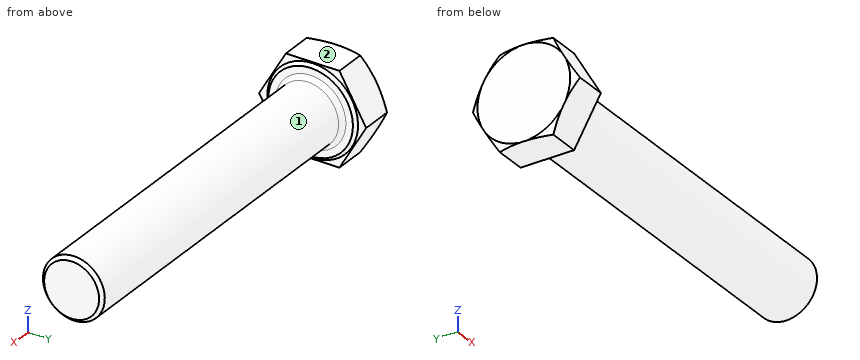
```python
from build123d import *

# Parameters (mm, degrees)
BOSS_EXTRUDE1_DEPTH = 7.5
SKETCH4_R           = 20.03
SKETCH4_R_2         = 9
CUT_EXTRUDE1_DEPTH  = 0.9375
CUT_EXTRUDE1_DRAFT  = -60
CHAMFER2_SIZE       = 0.666666667


with BuildPart() as part:
    # Sketch3 → Boss-Extrude1 (new body)
    with BuildSketch(Plane(origin=(0, 0, 0), x_dir=(0, 0, -1), z_dir=(1, 0, 0))):
        Polygon((9, 5.196152423), (0, 10.392304845), (-9, 5.196152423), (-9, -5.196152423), (0, -10.392304845), (9, -5.196152423), align=None)
    extrude(amount=BOSS_EXTRUDE1_DEPTH)


with BuildPart() as cut_extrude1_tool:
    # Sketch4 → Cut-Extrude1 (with draft: the straight prism first)
    with BuildSketch(Plane.ZY):
        Circle(SKETCH4_R)
        Circle(SKETCH4_R_2, mode=Mode.SUBTRACT)
    extrude(amount=-CUT_EXTRUDE1_DEPTH)
    # Cut-Extrude1: the draft: its side faces are tilted about the plane it starts from
    cut_extrude1_sides = [cut_extrude1_tool.faces().sort_by_distance(p)[0] for p in [
        (0.46875, 0, -20.03),
        (0.46875, 0, -9),
    ]]
    draft(cut_extrude1_sides, Plane.ZY, CUT_EXTRUDE1_DRAFT)


with BuildPart() as part_1:
    add(part.part)

    # Cut-Extrude1: cut by cut_extrude1_tool
    add(cut_extrude1_tool.part, mode=Mode.SUBTRACT)

    # Sketch5 → Revolve1 (revolve)
    with BuildSketch(Plane.XY, mode=Mode.PRIVATE) as revolve1_sk:
        with BuildLine():
            Line((8.35, 6), (77.5, 6))
            Line((77.5, 6), (77.5, 0))
            Line((77.5, 0), (7.5, 0))
            Line((7.5, 0), (7.5, 6.85))
            ThreePointArc((7.5, 6.85), (7.748959236, 6.248959236), (8.35, 6))
        make_face()
    revolve(revolve1_sk.sketch.rotate(Axis((7.5, 0, 0), (1, 0, 0)), 90), axis=Axis((7.5, 0, 0), (1, 0, 0)))

    # Chamfer2
    chamfer2_edges = [part_1.edges().sort_by_distance(p)[0] for p in [
        (77.5, 0, -6),
    ]]
    chamfer(chamfer2_edges, length=CHAMFER2_SIZE)

    # Sketch7 → Cut-Revolve1 (revolve, cut)
    with BuildSketch(Plane.XY, mode=Mode.PRIVATE) as cut_revolve1_sk:
        Polygon((7.5, 8.215), (6.9, 8.815), (6.9, 20.03), (7.5, 20.03), align=None)
    revolve(cut_revolve1_sk.sketch.rotate(Axis((0, 0, 0), (1, 0, 0)), 90), axis=Axis((0, 0, 0), (1, 0, 0)), mode=Mode.SUBTRACT)


solid = part_1.part
```
Build history of the part. All positions in model axes, mm. Face numbers are marked on the shaded views. A direction names the side the tool comes from. Round coordinates to 2 decimals unless told otherwise and drop trailing zeros. Write each loop counter-clockwise with the first axis right and the second up, starting at its lowest first coordinate (ties: lowest second). Pieces come first, ordered by that corner, then holes. Notation, with made-up numbers: (89, 52) -> (111, 52) arc R24 cw to (111, 62) -> close; hole circle Ø9 at (-22.75, 68). An arc over 180 degrees is marked (long way). Put each result on its own line as item: value.
Item 1: Slice it at A-A, the plane x = 15. Give the cut face in (y, z).
Here are the results:
outline: circle Ø12 at (0, 0)
Item 2: Wall check: probe 1 along X at (y, z) = (-7, 2); probe 2 along X at (y, z) = (5.75, -6.25); probe 3 along Y at (x, z) = (43, -4.5). Give the ranges that are in metal, low to high. Write a range as from..to.
Here are the results:
probe 1: x = 0..7.5
probe 2: x = 0..7.22
probe 3: y = -3.97..3.97
Item 3: Flat gauge pins, fed straight in: P1, Ø6, axis at x = 33.5, z = 2.5, coming from the -Y side; P2, Ø10, axis at x = 35.5, y = -6.5, coming from the +Z side; P3, Ø2, axis at x = 42, z = -3, coming from the -Y side; P4, Ø1.5, axis at x = 37.5, y = -8, coming from the +Z side. Where does each tip first touch, or does it go through?
Here are the results:
P1: stops at y = -6
P2: stops at z = 5.81
P3: stops at y = -5.66
P4: passes through
Item 4: Tool access for the marked faces 1 and 2: list every direction of +Z, -Z, +X, -X, +Y, -Y with a clear straight run to the whole face (end or side of a thin tool).
Here are the results:
face 1: +X
face 2: +Z, +X, -X, +Y, -Y
